Could you check a few things on this model? Use its own coordinates, in mm. Face numbers are marked on the shaded views. A direction names the side the tool comes from. Round coordinates to 2 decimals unless told otherwise and drop trailing zeros. Order: outer loops, then holes, each group sorted by start corner. A loop starts at its lowest first (then second) coordinate and runs counter-clockwise, first axis right, second up. Notation, with made-up numbers: M -27,-13 L 16,-13 A28 ccw 16,21 Z; hole C 88.25,80.25 d5. An arc over 180 degrees is marked long. Write each question's results on one line, items separated by ' | '. Start each with the question number.
1. I'm going to push flat-ended pins straight in: pin 1 (5 mm diameter, centred on x = 0, y = 47.5, fed in from -Z); pin 2 (1 mm diameter, centred on y = 27, z = 4, fed in from +X); pin 3 (1.6 mm diameter, centred on y = -1, z = 3.5, fed in from -X). Where does each tip first touch, or does it pass through?
2. Suppose I cut it at A-A on x = -59. Write out the boundary of the cut face in (y, z), and give its area (3 significant figures).
3. Suppose I cut it at C-C on y = 1. Write out the boundary of the cut face in (x, z), and give its area (3 significant figures).
4. Suppose I cut it at B-B on y = 47.5. Write out the boundary of the cut face in (x, z), and give its area (3 significant figures).
5. Please list where these lines run through material, in increasing order: L1, parallel to Y at x = 0, z = 1.95; L2, parallel to X at y = 47.5, z = 0.85; L3, parallel to Y at x = -23, z = -1.5.
6. Suppose I cut it at D-D on z = 1. Give the number of separate pieces and of enclosed holes in the cut face, and give its area (3 significant figures).
7. We'd pull the mould along X, two halves only. Please class the marked faces 4, 5, 6 and 7: released by +X, released by -X, zero draft, split by the parting line, or undercut.
8. For the marked faces 1, 2 and 3, which set-ups out of +Z, -Z, +X, -X, +Y, -Y let a thin tool reach every point of the face, with its end or its side?
from build123d import *

# Parameters (mm, degrees)
SKETCH1_W                                            = 130
SKETCH1_H                                            = 105
BOSS_EXTRUDE1_DEPTH                                  = 5
SKETCH3_R                                            = 22
CUT_EXTRUDE2_DEPTH                                   = 85.150163399
SKETCH7_W                                            = 30
SKETCH7_H                                            = 10
CUT_EXTRUDE5_DEPTH                                   = 15
FILLET1_R                                            = 6
CHAMFER1_SIZE                                        = 10
FILLET2_R                                            = 2
CUT_EXTRUDE8_DEPTH                                   = 85.150163399
FILLET3_R                                            = 2
CHAMFER2_SIZE                                        = 2
SKETCH15_W                                           = 1
SKETCH15_H                                           = 60.5
CUT_EXTRUDE10_DEPTH                                  = 85.150163399
HOLE_SIZE_PER_SOCKET_HEAD_CAP_SCREW_TYPE_D           = 4.5
HOLE_SIZE_PER_SOCKET_HEAD_CAP_SCREW_TYPE_CBORE_D     = 8
HOLE_SIZE_PER_SOCKET_HEAD_CAP_SCREW_TYPE_CBORE_DEPTH = 4.5
M3_TAPPED_HOLE1_D                                    = 2.5
M3_TAPPED_HOLE1_DEPTH                                = 8.5
M3_TAPPED_HOLE1_TIP                                  = 0.751075774
SKETCH20_W                                           = 1.5
SKETCH20_H                                           = 105
CUT_EXTRUDE11_DEPTH                                  = 2


with BuildPart() as part:
    # Sketch1 → Boss-Extrude1 (new, symmetric)
    with BuildSketch(Plane.XY):
        Rectangle(SKETCH1_W, SKETCH1_H)
    extrude(amount=BOSS_EXTRUDE1_DEPTH, both=True)

    # Sketch3 → Cut-Extrude2 (cut, through all)
    with BuildSketch(Plane.XY.offset(5)):
        with Locations((0, -62.5)):
            Circle(SKETCH3_R)
    extrude(amount=-CUT_EXTRUDE2_DEPTH, mode=Mode.SUBTRACT)

    # Sketch7 → Cut-Extrude5 (cut)
    with BuildSketch(Plane.XZ.offset(52.5)):
        with Locations((-50, 0)):
            Rectangle(SKETCH7_W, SKETCH7_H)
        with Locations((50, 0)):
            Rectangle(SKETCH7_W, SKETCH7_H)
    extrude(amount=-CUT_EXTRUDE5_DEPTH, mode=Mode.SUBTRACT)

    # Fillet1
    fillet1_edges = [part.edges().sort_by_distance(p)[0] for p in [
        (-35, -52.5, 0),
        (35, -52.5, 0),
    ]]
    fillet(fillet1_edges, radius=FILLET1_R)

    # Chamfer1
    chamfer1_edges = [part.edges().sort_by_distance(p)[0] for p in [
        (-65, -37.5, 0),
        (65, -37.5, 0),
    ]]
    chamfer(chamfer1_edges, length=CHAMFER1_SIZE)

    # Fillet2
    fillet2_edges = [part.edges().sort_by_distance(p)[0] for p in [
        (-35, -37.5, 0),
        (35, -37.5, 0),
    ]]
    fillet(fillet2_edges, radius=FILLET2_R)

    # Sketch10 → Cut-Extrude8 (cut, through all)
    with BuildSketch(Plane.XY.offset(5)):
        Polygon((-21.710710609, -31.184123297), (-17.436407821, -27.722861146), (-4.85, -43.265780375), (-9.124302788, -46.727042526), align=None)
    extrude(amount=-CUT_EXTRUDE8_DEPTH, mode=Mode.SUBTRACT)

    # Fillet3
    fillet3_edges = [part.edges().sort_by_distance(p)[0] for p in [
        (-19.595917942, -52.5, 0),
        (19.595917942, -52.5, 0),
    ]]
    fillet(fillet3_edges, radius=FILLET3_R)

    # Chamfer2
    chamfer2_edges = [part.edges().sort_by_distance(p)[0] for p in [
        (-65, 52.5, 0),
        (65, 52.5, 0),
    ]]
    chamfer(chamfer2_edges, length=CHAMFER2_SIZE)

    # Sketch15 → Cut-Extrude10 (cut, through all)
    with BuildSketch(Plane(origin=(0, 0, -5), x_dir=(-1, 0, 0), z_dir=(0, 0, -1))):
        with Locations((-64.5, 12.25)):
            Rectangle(SKETCH15_W, SKETCH15_H)
        with Locations((64.5, 12.25)):
            Rectangle(SKETCH15_W, SKETCH15_H)
    extrude(amount=-CUT_EXTRUDE10_DEPTH, mode=Mode.SUBTRACT)

    # Hole size per socket head cap screw type 0 (through all)
    with Locations(Plane(origin=(-18.523886338, 13.049633662, -5), x_dir=(1, 0, 0), z_dir=(0, 0, -1))):
        with Locations((77.523886338, -34.450366338), (18.523886338, -34.450366338), (-40.476113662, -34.450366338), (-40.476113662, 0.549633662), (-40.476113662, 35.549633662), (18.523886338, 40.549633662), (77.523886338, 35.549633662), (77.523886338, 0.549633662)):
            CounterBoreHole(HOLE_SIZE_PER_SOCKET_HEAD_CAP_SCREW_TYPE_D / 2, HOLE_SIZE_PER_SOCKET_HEAD_CAP_SCREW_TYPE_CBORE_D / 2, HOLE_SIZE_PER_SOCKET_HEAD_CAP_SCREW_TYPE_CBORE_DEPTH)

    # M3 Tapped Hole1
    with Locations(Plane(origin=(-15.568631127, 3.135719595, -5), x_dir=(1, 0, 0), z_dir=(0, 0, -1))):
        with Locations((-7.431368873, 28.635719595)):
            Hole(M3_TAPPED_HOLE1_D / 2, depth=M3_TAPPED_HOLE1_DEPTH)
            with Locations((0, 0, -(M3_TAPPED_HOLE1_DEPTH + M3_TAPPED_HOLE1_TIP / 2))):  # 118° drill point
                Cone(0, M3_TAPPED_HOLE1_D / 2, M3_TAPPED_HOLE1_TIP, mode=Mode.SUBTRACT)

    # Sketch20 → Cut-Extrude11 (cut)
    with BuildSketch(Plane.XY.offset(5)):
        Rectangle(SKETCH20_W, SKETCH20_H)
    extrude(amount=-CUT_EXTRUDE11_DEPTH, mode=Mode.SUBTRACT)


solid = part.part
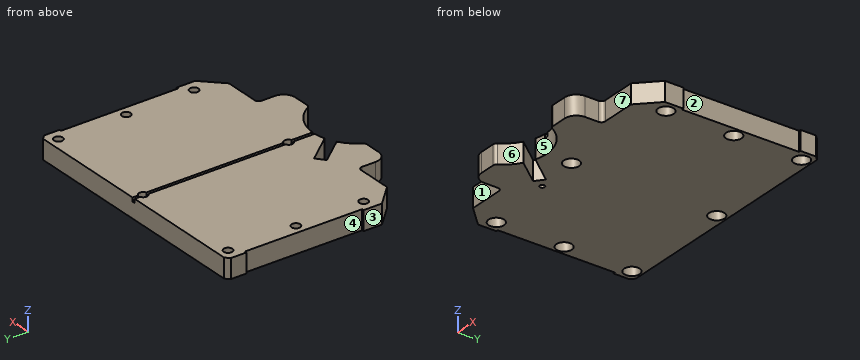
Filled sheet:
1) pin 1: stops at z = -0.5 | pin 2: stops at x = 64 | pin 3: stops at x = -64
2) outline: M -33.5,-5 L -26.5,-5 L -26.5,-0.5 L -24.75,-0.5 L -24.75,5 L -33.5,5 Z; M -20.25,-0.5 L -18.5,-0.5 L -18.5,-5 L 8.5,-5 L 8.5,-0.5 L 10.25,-0.5 L 10.25,5 L -20.25,5 Z; M 14.75,-0.5 L 16.5,-0.5 L 16.5,-5 L 43.5,-5 L 43.5,-0.5 L 45.25,-0.5 L 45.25,5 L 14.75,5 Z; M 49.75,-0.5 L 51.5,-0.5 L 51.5,-5 L 52.5,-5 L 52.5,5 L 49.75,5 Z | area: 678 mm^2
3) outline: M -64,-5 L 64,-5 L 64,5 L 0.75,5 L 0.75,3 L -0.75,3 L -0.75,5 L -64,5 Z | area: 1,280 mm^2
4) outline: M -65,-5 L -63,-5 L -63,-0.5 L -61.25,-0.5 L -61.25,5 L -65,5 Z; M -56.75,-0.5 L -55,-0.5 L -55,-5 L -4,-5 L -4,-0.5 L -2.25,-0.5 L -2.25,5 L -56.75,5 Z; M 2.25,-0.5 L 4,-0.5 L 4,-5 L 55,-5 L 55,-0.5 L 56.75,-0.5 L 56.75,5 L 2.25,5 Z; M 61.25,-0.5 L 63,-0.5 L 63,-5 L 65,-5 L 65,5 L 61.25,5 Z | area: 1,120 mm^2
5) L1: y = -40.5 to -29.75, -25.25 to 45.25, 49.75 to 52.5 | L2: x = -65 to -61.25, -56.75 to -2.25, 2.25 to 56.75, 61.25 to 65 | L3: y = -52.5 to -26.75, -24.25 to 52.5
6) separate pieces: 1 | enclosed holes: 9 | area: 12,000 mm^2
7) face 4: released by -X | face 5: undercut | face 6: undercut | face 7: zero draft
8) face 1: +Z, -Z, -X, -Y | face 2: +Z, -Z, +X | face 3: +Z, -Z, -X, +Y, -Y
